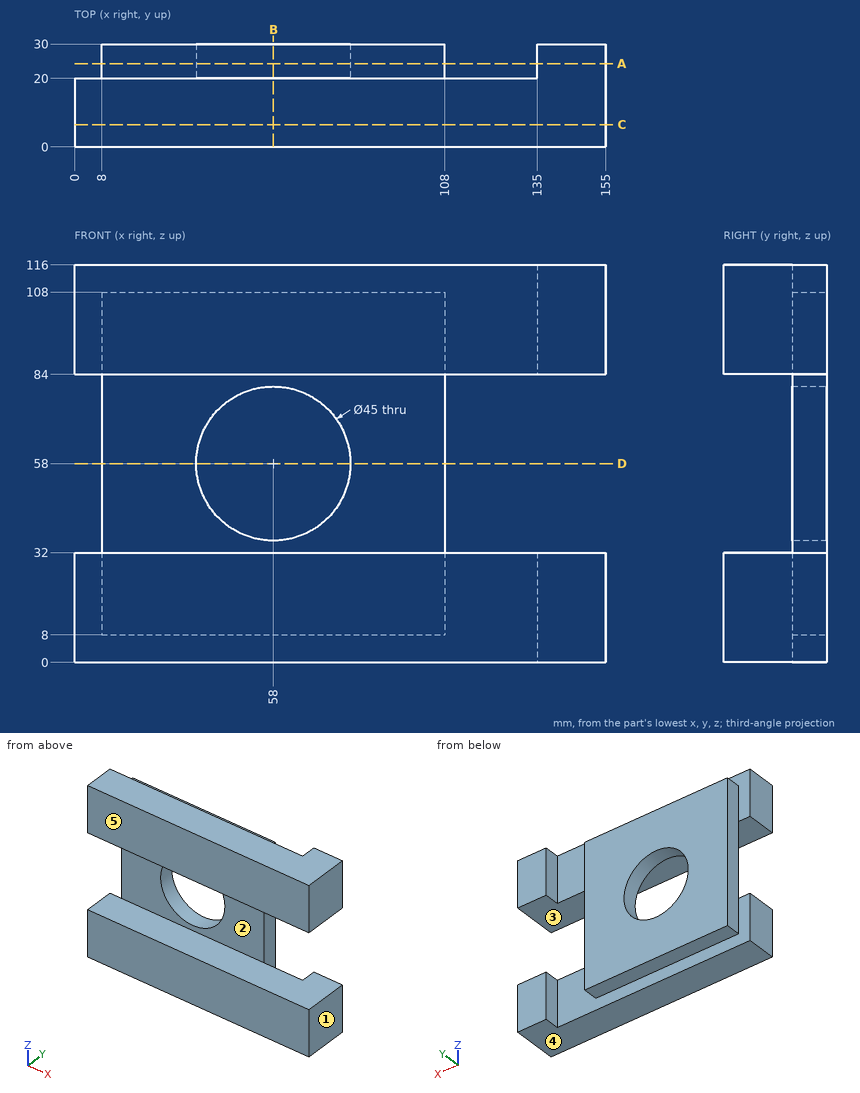
Answer from the drawing. Dimensions are ordinates in mm from the lowest x, y and z of the part. A direction names the side the tool comes from. Round coordinates to 2 decimals unless told otherwise and drop trailing zeros. Loops run counter-clockwise (first coordinate to the right, second up) from the corner with the lowest first, then second, coordinate; pieces in that order, holes last. Notation, with made-up numbers: (8.25, 5) - (20.25, 5) arc R31 cw to (20.25, 42) - close; hole circle Ø7 at (31.5, -14.75). An arc over 180 degrees is marked (long way). Return JSON: item names as keys, results as strings. Group by question number.
1. Each of these flat-tipped pins is pushed along its axis until it touches: P1, Ø8, axis at y = 27, z = 106.5, coming from the -X side; P2, Ø1, axis at x = 98.5, z = 68.5, coming from the -Y side; P3, Ø8, axis at y = 25, z = 53.5, coming from the +X side; P4, Ø10, axis at x = 65.5, z = 73, coming from the +Y side. Where does it stop, or does it pass through?
2. The part is cut by section B-B on x = 58. Determine the outline of the cut face in (y, z), then the cut area to 3 significant figures.
3. The part is cut by section D-D on z = 58. Determine the outline of the cut face in (x, y), then the cut area to 3 significant figures.
4. Which of the six approach directions +Z, -Z, +X, -X, +Y, -Y give full straight-line access (tool end or side, diameter ignored) to the marked faces 1 and 2?
5. The part is cut by section A-A on y = 24.25. Determine the outline of the cut face in (x, z).
6. Consider probe 1 along X at (y, z) = (26, 58); probe 2 along X at (y, z) = (27, 103); probe 3 along Z at (x, y) = (103.5, 16). Determine where each line is inside the solid, lowest interval first.
7. The mould has two halves that part along Z. Classify the marked faces 3, 4 and 5: pulls with the +Z half, pulls with the -Z half, needs draft (parallel to the pull), parting line crosses it, or undercut.
8. The part is cut by section C-C on y = 6.5. Determine the outline of the cut face in (x, z).
Resolved:
{
 "1": {"P1": "stops at x = 8", "P2": "stops at y = 20", "P3": "stops at x = 108", "P4": "passes through"},
 "2": {"outline": "(0, 0) - (20, 0) - (20, 8) - (30, 8) - (30, 35.5) - (20, 35.5) - (20, 32) - (0, 32) - close; (0, 84) - (20, 84) - (20, 80.5) - (30, 80.5) - (30, 108) - (20, 108) - (20, 116) - (0, 116) - close", "area": "1,830 mm²"},
 "3": {"outline": "(8, 20) - (35.5, 20) - (35.5, 30) - (8, 30) - close; (80.5, 20) - (108, 20) - (108, 30) - (80.5, 30) - close", "area": "550 mm²"},
 "4": {"face 1": "+Z, -Z, +X, +Y, -Y", "face 2": "+X, -X, -Y"},
 "5": {"outline": "(8, 8) - (108, 8) - (108, 108) - (8, 108) - close; (135, 0) - (155, 0) - (155, 32) - (135, 32) - close; (135, 84) - (155, 84) - (155, 116) - (135, 116) - close; hole circle Ø45 at (58, 58)"},
 "6": {"probe 1": "x = 8 to 35.5, 80.5 to 108", "probe 2": "x = 8 to 108, 135 to 155", "probe 3": "z = 0 to 32, 84 to 116"},
 "7": {"face 3": "undercut", "face 4": "pulls with the -Z half", "face 5": "needs draft"},
 "8": {"outline": "(0, 0) - (155, 0) - (155, 32) - (0, 32) - close; (0, 84) - (155, 84) - (155, 116) - (0, 116) - close"}
}
